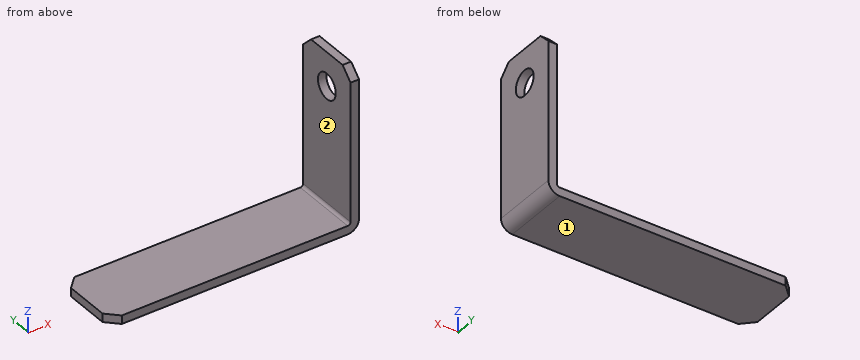
```python
from build123d import *

# Parameters (mm, degrees)
BOSS_EXTRUDE1_DEPTH = 12
SKETCH2_R           = 2.25
CUT_EXTRUDE1_DEPTH  = 54.779642989
CHAMFER1_SIZE       = 2
FILLET1_R           = 2
FILLET2_R           = 0.5


with BuildPart() as part:
    # Sketch1 → Boss-Extrude1 (new body)
    with BuildSketch(Plane(origin=(0, 0, 0), x_dir=(1, 0, 0), z_dir=(0, 1, 0))):
        Polygon((0, 0), (-1.5, 0), (-1.5, 27), (-44, 27), (-44, 28.5), (0, 28.5), align=None)
    extrude(amount=BOSS_EXTRUDE1_DEPTH)

    # Sketch2 → Cut-Extrude1 (cut, through all)
    with BuildSketch(Plane(origin=(0, 0, 0), x_dir=(0, 0, -1), z_dir=(1, 0, 0))):
        with Locations((6, 6)):
            Circle(SKETCH2_R)
    extrude(amount=-CUT_EXTRUDE1_DEPTH, mode=Mode.SUBTRACT)

    # Chamfer1
    chamfer1_edges = [part.edges().sort_by_distance(p)[0] for p in [
        (-44, 12, -27.75),
        (-0.75, 12, 0),
        (-0.75, 0, 0),
        (-44, 0, -27.75),
    ]]
    chamfer(chamfer1_edges, length=CHAMFER1_SIZE)

    # Fillet1
    fillet1_edges = [part.edges().sort_by_distance(p)[0] for p in [
        (0, 6, -28.5),
    ]]
    fillet(fillet1_edges, radius=FILLET1_R)

    # Fillet2
    fillet2_edges = [part.edges().sort_by_distance(p)[0] for p in [
        (-1.5, 6, -27),
    ]]
    fillet(fillet2_edges, radius=FILLET2_R)


solid = part.part
```
Here's how the part is built. I have some questions about the finished solid (model axes, mm). Face numbers are marked on the shaded views. A direction names the side the tool comes from. Round coordinates to 2 decimals unless told otherwise and drop trailing zeros. Loops run counter-clockwise (first coordinate to the right, second up) from the corner with the lowest first, then second, coordinate; pieces in that order, holes last. Notation, with made-up numbers: (89, -31) -> (145, -31) arc R31 cw to (145, 0) -> close; hole circle Ø10 at (11.25, 13.25). An arc over 180 degrees is marked (long way). Answer as CSV lines item,"result". Start each with the question number.
1. Imagine slicing it at C-C on y = 6. Write out the boundary of the cut face in (x, z), plus the area to 3 significant figures.
2. Imagine slicing it at B-B on y = 11.25. Write out the boundary of the cut face in (x, z).
3. Imagine slicing it at A-A on z = -6. Write out the boundary of the cut face in (x, y), plus the area to 4 significant figures.
4. For the marked faces 1 and 2, which set-ups out of +Z, -Z, +X, -X, +Y, -Y let a thin tool reach every point of the face, with its end or its side?
5. I'm going to push a flat-ended pin straight in: P1, Ø3, axis at y = 2.5, z = -9, coming from the -X side. Where does the tip first touch, or does it pass through?
6. I need wall thicknesses on probe 1 along Y at (x, z) = (-0.25, -6); probe 2 along X at (y, z) = (5.5, -14); probe 3 along Z at (x, y) = (-3, 10.5). Which ranges of each line are inside material? Lowest first, please. Write a range as from..to.
7. Imagine slicing it at D-D on x = -4. Write out the boundary of the cut face in (y, z).
Solution:
1,outline,"(-44, -28.5) -> (-2, -28.5) arc R2 ccw to (0, -26.5) -> (0, -8.25) -> (-1.5, -8.25) -> (-1.5, -26.5) arc R0.5 cw to (-2, -27) -> (-44, -27) -> close; (-1.5, -3.75) -> (0, -3.75) -> (0, 0) -> (-1.5, 0) -> close"
1,area,"98.9 mm²"
2,outline,"(-42.75, -28.5) -> (-2, -28.5) arc R2 ccw to (0, -26.5) -> (0, -1.25) -> (-1.5, -1.25) -> (-1.5, -26.5) arc R0.5 cw to (-2, -27) -> (-42.75, -27) -> close"
3,outline,"(-1.5, 0) -> (0, 0) -> (0, 3.75) -> (-1.5, 3.75) -> close; (-1.5, 8.25) -> (0, 8.25) -> (0, 12) -> (-1.5, 12) -> close"
3,area,"11.25 mm²"
4,face 1,"-Z, +X, -X, +Y, -Y"
4,face 2,"+Z, -X, +Y, -Y"
5,P1,"x = -1.5"
6,probe 1,"0..3.75, 8.25..12"
6,probe 2,"-1.5..0"
6,probe 3,"-28.5..-27"
7,outline,"(0, -28.5) -> (12, -28.5) -> (12, -27) -> (0, -27) -> close"
